Design review of the part shown in the three views and the two pictorial views. Dimensions are in mm from the part's minimum x, y and z. A direction names the side the tool comes from. Coordinates: 2 decimals unless noted, no trailing zeros. Order: outer loops, then holes, each group sorted by start corner. A loop starts at its lowest first (then second) coordinate and runs counter-clockwise, first axis right, second up. Notation, with made-up numbers: (-5.75, 18) - (14.25, 18) arc R4 cw to (14.25, 25) - close; hole circle Ø8 at (22.5, -31). An arc over 180 degrees is marked (long way). One line per item, written item: value. Start each with the question number.
(1) Consider section B-B on z = 100. Write out the cut boundary in (x, y), then the cut area to 3 significant figures.
(2) Consider section A-A on y = 10. Write out the cut boundary in (x, z), then the cut area to 3 significant figures.
(3) To check wall thickness, follow line 1 along X through (y, z) = (13.5, 20); line 2 along X through (y, z) = (2.95, 20); line 3 along Z through (x, y) = (12.5, 2.3). State the ranges of each line that lie inside material, in increasing order.
(4) Clearance check with flat-ended pins moving along their axes: pin 1 (19.5 mm diameter, centred on x = 12.5, z = 100, fed in from +Y); pin 2 (8 mm diameter, centred on y = 10, z = 60, fed in from +X). State where each tip first meets the part, or that it passes through.
(5) Consider section D-D on z = 45.5. Write out the cut boundary in (x, y), then the cut area to 3 significant figures.
(6) For the marked faces 1, 2 and 3, list the 3-axis set-ups (+Z, -Z, +X, -X, +Y, -Y) from which the entire face can be reached by the end or side of a thin tool; tool diameter is ignored.
(7) Mouldability with a two-part tool opening along X and no side actions: class the marked faces 4, 5 and 6 as released by +X, released by -X, zero draft, split by the parting line, or undercut.
(8) Consider section C-C on x = 72.5. Write out the cut boundary in (y, z).
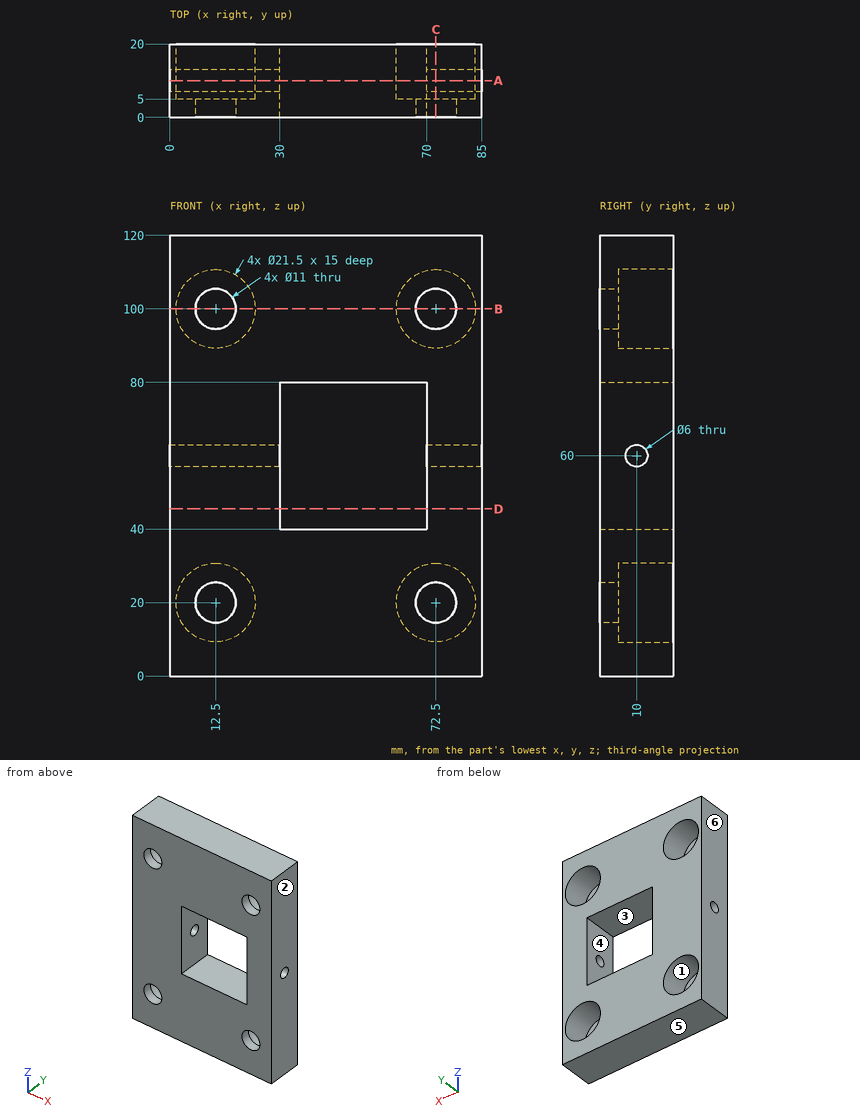
Geometry check:
1. outline: (0, 0) - (7, 0) - (7, 5) - (1.75, 5) - (1.75, 20) - (0, 20) - close; (18, 0) - (67, 0) - (67, 5) - (61.75, 5) - (61.75, 20) - (23.25, 20) - (23.25, 5) - (18, 5) - close; (78, 0) - (85, 0) - (85, 20) - (83.25, 20) - (83.25, 5) - (78, 5) - close
1. area: 945 mm^2
2. outline: (0, 0) - (85, 0) - (85, 57) - (70, 57) - (70, 40) - (30, 40) - (30, 57) - (0, 57) - close; (0, 63) - (30, 63) - (30, 80) - (70, 80) - (70, 63) - (85, 63) - (85, 120) - (0, 120) - close; hole circle Ø21.5 at (12.5, 20); hole circle Ø21.5 at (12.5, 100); hole circle Ø21.5 at (72.5, 20); hole circle Ø21.5 at (72.5, 100)
2. area: 6,880 mm^2
3. line 1: x = 0 to 1.75, 23.25 to 61.75, 83.25 to 85
3. line 2: x = 0 to 7, 18 to 67, 78 to 85
3. line 3: z = 0 to 14.5, 25.5 to 94.5, 105.5 to 120
4. pin 1: stops at y = 5
4. pin 2: stops at x = 85
5. outline: (0, 0) - (30, 0) - (30, 20) - (0, 20) - close; (70, 0) - (85, 0) - (85, 20) - (70, 20) - close
5. area: 900 mm^2
6. face 1: +Y
6. face 2: +Z, -Z, +X, +Y, -Y
6. face 3: +Y, -Y
7. face 4: undercut
7. face 5: zero draft
7. face 6: released by -X
8. outline: (0, 0) - (20, 0) - (20, 9.25) - (5, 9.25) - (5, 14.5) - (0, 14.5) - close; (0, 25.5) - (5, 25.5) - (5, 30.75) - (20, 30.75) - (20, 89.25) - (5, 89.25) - (5, 94.5) - (0, 94.5) - close; (0, 105.5) - (5, 105.5) - (5, 110.75) - (20, 110.75) - (20, 120) - (0, 120) - close; hole circle Ø6 at (10, 60)
